Source: three-view drawing plus pictorial views. Frame: mm from the lowest corner of the part. Coordinates: 2 decimals unless noted, no trailing zeros. Write each loop counter-clockwise with the first axis right and the second up, starting at its lowest first coordinate (ties: lowest second). Pieces come first, ordered by that corner, then holes. Notation, with made-up numbers: (19.25, 21) -> (49.25, 21) arc R20 ccw to (49.25, 30) -> close; hole circle Ø2 at (47.5, -36.5). An arc over 180 degrees is marked (long way). One line per question, with ' | ' between items. Start each with the question number.
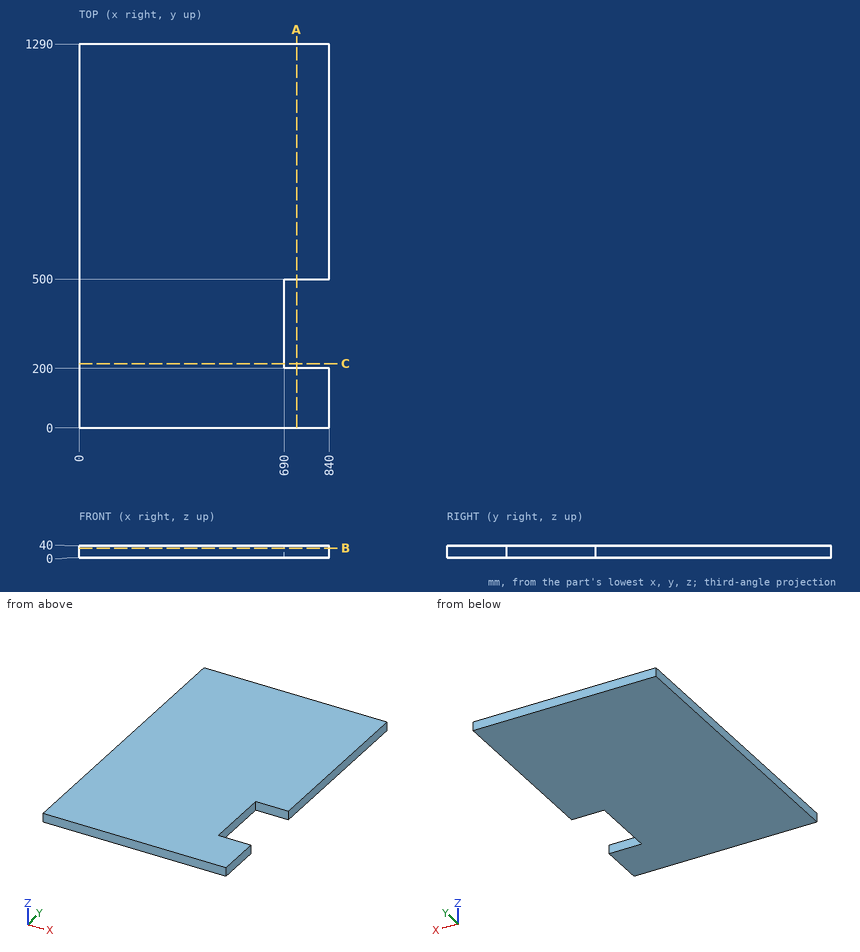
1) Section A-A, the plane x = 731. Return loops of the section in (y, z), then the cut area to 3 significant figures.
2) Ray query, line 1 (Y direction, x = 758, z = 23.5); line 2 (X direction, y = 327, z = 22). Return the intervals inside material, ascending.
3) Section B-B, the plane z = 32.5. Return loops of the section in (x, y), then the cut area to 3 significant figures.
4) Section C-C, the plane y = 216. Return loops of the section in (x, z), then the cut area to 3 significant figures.
Answer block:
1) outline: (0, 0) -> (200, 0) -> (200, 40) -> (0, 40) -> close; (500, 0) -> (1290, 0) -> (1290, 40) -> (500, 40) -> close | area: 39,600 mm2
2) line 1: y = 0 to 200, 500 to 1290 | line 2: x = 0 to 690
3) outline: (0, 0) -> (840, 0) -> (840, 200) -> (690, 200) -> (690, 500) -> (840, 500) -> (840, 1290) -> (0, 1290) -> close | area: 1,040,000 mm2
4) outline: (0, 0) -> (690, 0) -> (690, 40) -> (0, 40) -> close | area: 27,600 mm2
